from build123d import *

# Parameters (mm, degrees)
SKETCH1_W           = 1200
SKETCH1_H           = 415
BOSS_EXTRUDE1_DEPTH = 20
SKETCH2_W           = 10
SKETCH2_H           = 40
CUT_EXTRUDE1_DEPTH  = 280


with BuildPart() as part:
    # Sketch1 → Boss-Extrude1 (new body)
    with BuildSketch(Plane.XY):
        with Locations((600, 207.5)):
            Rectangle(SKETCH1_W, SKETCH1_H)
    extrude(amount=BOSS_EXTRUDE1_DEPTH)

    # Sketch2 → Cut-Extrude1 (cut)
    with BuildSketch(Plane.XY.offset(20)):
        with Locations((5, 395)):
            Rectangle(SKETCH2_W, SKETCH2_H)
        with Locations((1195, 395)):
            Rectangle(SKETCH2_W, SKETCH2_H)
        with Locations((1195, 20)):
            Rectangle(SKETCH2_W, SKETCH2_H)
        with Locations((5, 20)):
            Rectangle(SKETCH2_W, SKETCH2_H)
    extrude(amount=-CUT_EXTRUDE1_DEPTH, mode=Mode.SUBTRACT)


solid = part.part
Source: CAD feature listing. Evaluate the final solid. Frame: model axes, mm. A direction names the side the tool comes from. Round coordinates to 2 decimals unless told otherwise and drop trailing zeros. Write each loop counter-clockwise with the first axis right and the second up, starting at its lowest first coordinate (ties: lowest second). Pieces come first, ordered by that corner, then holes. Notation, with made-up numbers: (-16.75, 27.25) - (29.25, 27.25) arc R32 ccw to (29.25, 58.25) - close; hole circle Ø9 at (78.5, 1). An arc over 180 degrees is marked (long way). Use CSV: the item, a comma, the result in double quotes. Start each with the question number.
(1) Cut plane A-A, the plane y = 29.5. Return loops of the section in (x, z).
(2) First-contact query: pin 1 Ø3 at (x, z) = (7, 10.5) entering from -Y; pin 2 Ø6 at (y, z) = (28, 12.5) entering from -X; pin 3 Ø5 at (x, z) = (1194, 12.5) entering from +Y. Flat tips, straight axial feed; report the tip coordinate or a pass-through.
(3) Set-up query: faces 1 (the face through (10, 20, 10)), 2 (the face through (1190, 20, 10)), 3 (the face through (10, 395, 10)). Return all of +Z, -Z, +X, -X, +Y, -Y with unobstructed straight access to the full face (end or side cutting, diameter ignored); none if empty.
Geometry says:
1,outline,"(10, 0) - (1190, 0) - (1190, 20) - (10, 20) - close"
2,pin 1,"y = 40"
2,pin 2,"x = 10"
2,pin 3,"y = 375"
3,face 1,"+Z, -Z, -X, -Y"
3,face 2,"+Z, -Z, +X, -Y"
3,face 3,"+Z, -Z, -X, +Y"
